Source: CAD feature listing. Evaluate the final solid. Frame: model axes, mm. A direction names the side the tool comes from. Give positions to 0.01 mm unless a question says otherwise; leave off trailing zeros. Loops run counter-clockwise (first coordinate to the right, second up) from the corner with the lowest first, then second, coordinate; pieces in that order, holes last. Notation, with made-up numbers: M 12.25,-30 L 30.25,-30 A22 cw 30.25,-4 Z; hole C 34,0 d11. An arc over 180 degrees is marked long. Answer in a Markdown table with one row per item.
```python
from build123d import *

# Parameters (mm, degrees)
BRACKET_BODY_DEPTH          = 55
WEB_START                   = -27.5
WEB_BOSS_180X70_DEPTH       = 5
WEB_BOSS_74_DEPTH           = 5
HUB_BOSS_SKETCH_R           = 26
HUB_BOSS_DEPTH              = 55
ANGLED_CUT_30DEG_DEPTH      = 55
BEND_FILLETS_R20_R          = 20
HUB_SUPPORT_RIB_REACH       = 218.543
SUPPORT_RIB_SKETCH_WALL_W   = 572.021051398
SUPPORT_RIB_SKETCH_WALL_H   = 10
HUB_BORE_SKETCH_R           = 16
HUB_BORE_32_DEPTH           = 55
FLANGE_HOLES_SKETCH_R       = 5.5
FLANGE_HOLES_SKETCH_R_2     = 4.5
FLANGE_MOUNTING_HOLES_DEPTH = 55
EDGE_FILLETS_R5_R           = 5
WEB_FILLETS_R5_R            = 5
CROSS_HOLE_SKETCH_R         = 5
HUB_CROSS_HOLE_10_DEPTH     = 45


with BuildPart() as part:
    # Bracket Profile Sketch → Bracket Body (new body)
    with BuildSketch(Plane.XY):
        Polygon((0, 0), (155, 0), (172.25, 23), (205.25, 23), (205.25, 35), (168.75, 35), (150, 10), (5, 10), (-13.75, 35), (-50.25, 35), (-50.25, 23), (-17.25, 23), align=None)
    extrude(amount=-BRACKET_BODY_DEPTH)

    # Web Boss 180x70 Sketch → Web Boss 180x70 (add, symmetric)
    with BuildSketch(Plane.XY.offset(WEB_START)):
        Polygon((-12.25, 33), (7, 33), (77, 10), (5, 10), align=None)
    extrude(amount=WEB_BOSS_180X70_DEPTH, both=True)

    # Web Boss 74 Sketch → Web Boss 74 (add, symmetric)
    with BuildSketch(Plane.XY.offset(WEB_START)):
        Polygon((167.25, 33), (114.75, 10), (150, 10), align=None)
    extrude(amount=WEB_BOSS_74_DEPTH, both=True)

    # Hub Boss Sketch → Hub Boss (add)
    with BuildSketch(Plane.XY):
        with Locations((134.75, -37.3)):
            Circle(HUB_BOSS_SKETCH_R)
        with BuildLine():
            ThreePointArc((129.75, -11.785298356), (134.75, -11.3), (139.75, -11.785298356))
            Line((139.75, -11.785298356), (139.75, 0))
            Line((139.75, 0), (129.75, 0))
            Line((129.75, 0), (129.75, -11.785298356))
        make_face()
    extrude(amount=-HUB_BOSS_DEPTH)

    # Angled Cut Sketch → Angled Cut 30deg (cut)
    with BuildSketch(Plane(origin=(0, 35, 0), x_dir=(1, 0, 0), z_dir=(0, 1, 0))):
        Polygon((-50.25, 55), (-50.25, 22.567969878), (-34.99199027, 55), align=None)
        Polygon((-37.220376516, 0), (-50.25, 22.567969878), (-50.25, 0), align=None)
    extrude(amount=-ANGLED_CUT_30DEG_DEPTH, mode=Mode.SUBTRACT)

    # Bend Fillets R20
    bend_fillets_r20_edges = [part.edges().sort_by_distance(p)[0] for p in [
        (5, 10, -43.75),
        (150, 10, -43.75),
        (155, 0, -27.5),
        (0, 0, -27.5),
        (5, 10, -11.25),
        (150, 10, -11.25),
    ]]
    fillet(bend_fillets_r20_edges, radius=BEND_FILLETS_R20_R)

    # Support Rib Sketch wall → Hub Support Rib (add, up to next)
    with BuildSketch(Plane(origin=(61.965504267, -29.159208524, -27.5), x_dir=(0.889610508712, -0.45671998291, 0), z_dir=(0.45671998291, 0.889610508712, 0)), mode=Mode.PRIVATE) as hub_support_rib_sk1:
        Rectangle(SUPPORT_RIB_SKETCH_WALL_W, SUPPORT_RIB_SKETCH_WALL_H)
    hub_support_rib_tool1 = extrude(hub_support_rib_sk1.sketch, amount=HUB_SUPPORT_RIB_REACH, mode=Mode.PRIVATE) - part.part
    add(hub_support_rib_tool1.solids().sort_by_distance((61.965504267, -29.159208524, -27.5))[0])

    # Hub Bore Sketch → Hub Bore Ø32 (cut)
    with BuildSketch(Plane.XY):
        with Locations((134.75, -37.3)):
            Circle(HUB_BORE_SKETCH_R)
    extrude(amount=-HUB_BORE_32_DEPTH, mode=Mode.SUBTRACT)

    # Flange Holes Sketch → Flange Mounting Holes (cut)
    with BuildSketch(Plane(origin=(0, 35, 0), x_dir=(1, 0, 0), z_dir=(0, 1, 0))):
        with Locations(Location((-34.024558742, 22.967597982, 0), (0, 0, 180))):
            Circle(FLANGE_HOLES_SKETCH_R)
        with Locations(Location((-26, 43.020043273, 0), (0, 0, 180))):
            Circle(FLANGE_HOLES_SKETCH_R_2)
        with Locations(Location((186.25, 42.5, 0), (0, 0, 180))):
            Circle(FLANGE_HOLES_SKETCH_R)
        with Locations(Location((186.25, 27.5, 0), (0, 0, 180))):
            Circle(FLANGE_HOLES_SKETCH_R_2)
        with Locations(Location((186.25, 12.5, 0), (0, 0, 180))):
            Circle(FLANGE_HOLES_SKETCH_R)
    extrude(amount=-FLANGE_MOUNTING_HOLES_DEPTH, mode=Mode.SUBTRACT)

    # Edge Fillets R5
    edge_fillets_r5_edges = [part.edges().sort_by_distance(p)[0] for p in [
        (205.25, 29, 0),
        (205.25, 29, -55),
    ]]
    fillet(edge_fillets_r5_edges, radius=EDGE_FILLETS_R5_R)

    # Web Fillets R5
    web_fillets_r5_edges = [part.edges().sort_by_distance(p)[0] for p in [
        (161.625, 25.5, -22.5),
        (161.625, 25.5, -32.5),
        (148.94427191, 12.11145618, -32.5),
        (46, 10, -32.5),
        (46, 10, -22.5),
        (148.94427191, 12.11145618, -22.5),
        (6.05572809, 12.11145618, -32.5),
        (6.05572809, 12.11145618, -22.5),
        (-6.625, 25.5, -32.5),
        (-6.625, 25.5, -22.5),
        (127.375, 10, -32.5),
        (127.375, 10, -22.5),
    ]]
    fillet(web_fillets_r5_edges, radius=WEB_FILLETS_R5_R)

    # Cross Hole Sketch → Hub Cross Hole Ø10 (cut)
    with BuildSketch(Plane(origin=(163.566905934, -8.483094066, 0), x_dir=(0.7071067811865488, -0.7071067811865462, 0), z_dir=(0.7071067811865462, 0.7071067811865488, 0))):
        with Locations(Location((0.493915353, 27.5, 0), (0, 0, 180))):
            Circle(CROSS_HOLE_SKETCH_R)
    extrude(amount=-HUB_CROSS_HOLE_10_DEPTH, mode=Mode.SUBTRACT)


solid = part.part
```
Q1. Section query B-B (x = -26). Output: boundary loops of the cut face in (y, z), plus the area to 3 significant figures.
Values follow:
| item | result |
|---|---|
| outline | M 23,-55 L 35,-55 L 35,-47.52 L 23,-47.52 Z; M 23,-38.52 L 35,-38.52 L 35,0 L 23,0 Z |
| area | 552 mm^2 |
Q2. Section query D-D (x = 186.25). Output: boundary loops of the cut face in (y, z).
Values follow:
| item | result |
|---|---|
| outline | M 23,-55 L 35,-55 L 35,-48 L 23,-48 Z; M 23,-37 L 35,-37 L 35,-32 L 23,-32 Z; M 23,-23 L 35,-23 L 35,-18 L 23,-18 Z; M 23,-7 L 35,-7 L 35,0 L 23,0 Z |
Q3. Section query A-A (y = -37.3). Output: boundary loops of the cut face in (x, z), plus the area to 3 significant figures.
Values follow:
| item | result |
|---|---|
| outline | M 77.82,-32.5 L 108.75,-32.5 L 108.75,-55 L 118.75,-55 L 118.75,0 L 108.75,0 L 108.75,-22.5 L 77.82,-22.5 Z; M 150.75,-55 L 160.75,-55 L 160.75,0 L 150.75,0 Z |
| area | 1,410 mm^2 |
Q4. Ray query, probe 1 along Z at (x, y) = (186.25, 32.5); probe 2 along Y at (x, z) = (128, -6.5); probe 3 along X at (y, z) = (-37.5, -3). Return the intervals inside material, ascending. Write a range as from..to.
Values follow:
| item | result |
|---|---|
| probe 1 | -55..-48, -37..-32, -23..-18, -7..0 |
| probe 2 | -62.41..-51.81, -22.79..-12.19, 0..10 |
| probe 3 | 108.75..118.75, 150.75..160.75 |
Q5. Contact query for flat-ended pins moving along their axis: pin 1 Ø4 at (x, z) = (-12, -24.5) entering from +Y; pin 2 Ø3 at (x, y) = (9, 15) entering from +Z; pin 3 Ø12 at (y, z) = (-24, -6) entering from +X; pin 4 Ø7 at (x, z) = (186.25, -27.5) entering from -Y. Output: stop coordinate, or through.
Values follow:
| item | result |
|---|---|
| pin 1 | y = 35 |
| pin 2 | z = -21.74 |
| pin 3 | x = 159.7 |
| pin 4 | through |
Q6. Section query C-C (z = -12.5). Output: boundary loops of the cut face in (x, y).
Values follow:
| item | result |
|---|---|
| outline | M -44.44,23 L -17.25,23 L -6,8 A20 ccw 10,0 L 129.75,0 L 129.75,-11.79 A26 ccw long 139.75,-11.79 L 139.75,0 L 145,0 A20 ccw 161,8 L 172.25,23 L 180.75,23 L 180.75,35 L 168.75,35 L 156,18 A20 cw 140,10 L 15,10 A20 cw -1,18 L -13.75,35 L -44.44,35 Z; M 191.75,23 L 205.25,23 L 205.25,35 L 191.75,35 Z; hole C 134.75,-37.3 d32 |
Q7. Mould query, pull axis Y, two halves, no side actions, for faces 1 (the flat face through (129.75, -6, -11)), 2 (the cylindrical face through (148.828, 12.054, -46.372)), 3 (the cylindrical face through (-0.63, 3.06, -27.88)). Classes: +Y half, -Y half, draft (parallel to the pull), parting line (faces both ways), or undercut.
Values follow:
| item | result |
|---|---|
| face 1 | undercut |
| face 2 | +Y half |
| face 3 | -Y half |
Q8. Reachability of faces 4 (the flat face through (69, 0, -11)), 5 (the cylindrical face through (149.73, -58.55, -27.12)), 6 (the cylindrical face through (148.828, 12.054, -8.872)), 7 (the flat face through (41.51, 21.66, -27.36)), 8 (the flat face through (142, 0, -27)) from +Z, -Z, +X, -X, +Y, -Y: full face, straight path, thin tool, end or side. Return the list, or none.
Values follow:
| item | result |
|---|---|
| face 4 | +Z, -X |
| face 5 | none |
| face 6 | +Z, +Y |
| face 7 | +Z, -Z, +Y |
| face 8 | +Z, -Z, +X |
